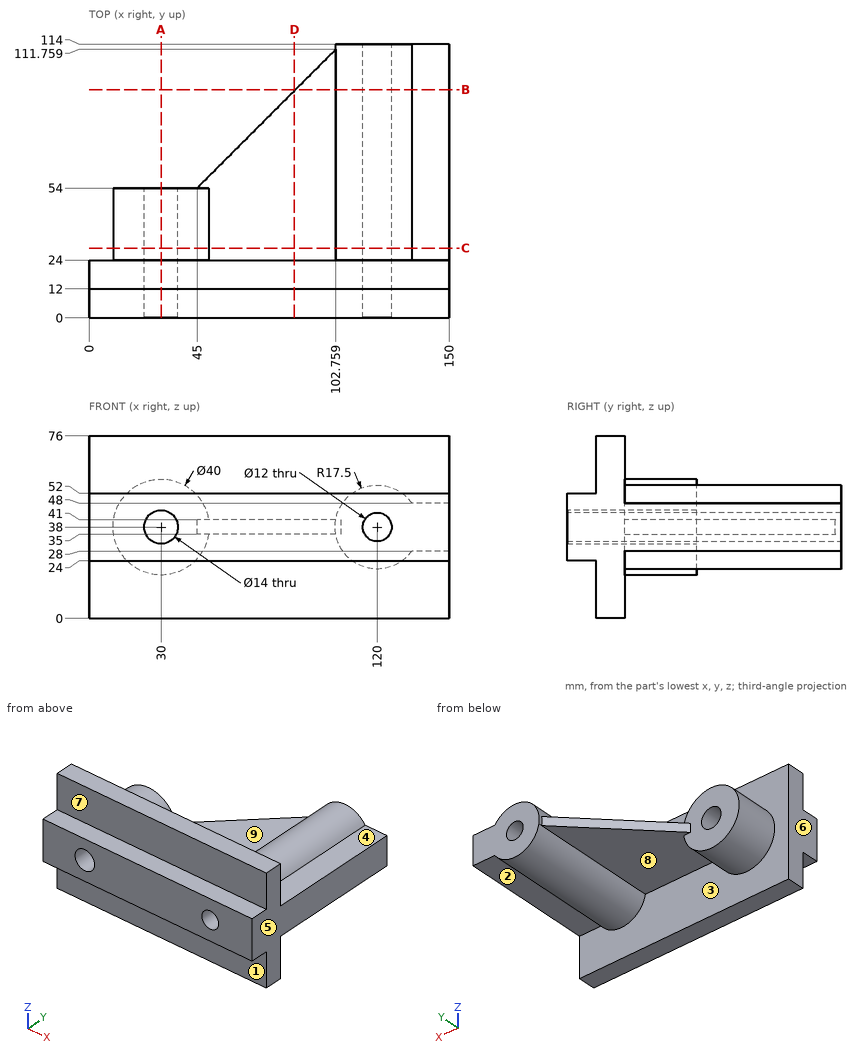
Could you check a few things on this drawing? It's one solid part, dimensions in mm from its lowest x, y, z. A direction names the side the tool comes from. Give positions to 0.01 mm unless a question says otherwise; leave off trailing zeros. Loops run counter-clockwise (first coordinate to the right, second up) from the corner with the lowest first, then second, coordinate; pieces in that order, holes last. Notation, with made-up numbers: M 3,56 L 42,56 A18 ccw 42,88 Z; hole C 2.5,-26 d6. An arc over 180 degrees is marked long. One line per question, with ' | ' between items. Start each with the question number.
Q1. If I drill on line 1 (X direction, y = 13, z = 38); line 2 (X direction, y = 30, z = 38); line 3 (X direction, y = 67, z = 38), over which ranges is the centre line in solid material (lowest first)? Write a range as from..to.
Q2. If we section it at C-C (y = 29): Please give me the cut outline in (x, z), plus the area to 3 significant figures.
Q3. For pin 1 Ø12 at (y, z) = (92.5, 20.5) entering from -X; pin 2 Ø17.5 at (x, y) = (73, 47.5) entering from +Z; pin 3 Ø19 at (x, z) = (93, 8.5) entering from -Y, each with a flat end and sliding along its axis, tell me the tip position at first contact or that it passes through.
Q4. If we section it at A-A (x = 30): Please give me the cut outline in (y, z), plus the area to 3 significant figures.
Q5. If we section it at D-D (x = 85.5): Please give me the cut outline in (y, z).
Q6. If we section it at B-B (y = 95): Please give me the cut outline in (x, z), plus the area to 3 significant figures.
Q7. If we mould it in two halves opening along X, with no side actions, what happens to the marked faces 6, 7, 8 and 9? For each: +X half, -X half, draft (parallel to the pull), parting line (faces both ways), or undercut.
Q8. For the marked faces 1, 2, 3, 4 and 5, which set-ups out of +Z, -Z, +X, -X, +Y, -Y let a thin tool reach every point of the face, with its end or its side?
Computed:
1) line 1: x = 0..23, 37..114, 126..150 | line 2: x = 10..23, 37..114, 126..150 | line 3: x = 58..114, 126..150
2) outline: M 49.77,35 L 102.76,35 A17.5 ccw 134.36,28 L 150,28 L 150,48 L 134.36,48 A17.5 ccw 102.76,41 L 49.77,41 A20 ccw long Z; hole C 30,38 d14; hole C 120,38 d12 | area: 2,540 mm²
3) pin 1: stops at x = 106.81 | pin 2: stops at z = 41 | pin 3: stops at y = 12
4) outline: M 0,24 L 12,24 L 12,0 L 24,0 L 24,18 L 54,18 L 54,31 L 0,31 Z; M 0,45 L 54,45 L 54,58 L 24,58 L 24,76 L 12,76 L 12,52 L 0,52 Z | area: 1,690 mm²
5) outline: M 0,24 L 12,24 L 12,0 L 24,0 L 24,35 L 94.5,35 L 94.5,41 L 24,41 L 24,76 L 12,76 L 12,52 L 0,52 Z
6) outline: M 86,35 L 102.76,35 A17.5 ccw 134.36,28 L 150,28 L 150,48 L 134.36,48 A17.5 ccw 102.76,41 L 86,41 Z; hole C 120,38 d12 | area: 1,220 mm²
7) face 6: -X half | face 7: draft | face 8: undercut | face 9: undercut
8) face 1: -Z, +X, -X, -Y | face 2: -Z, +X, +Y | face 3: +Y | face 4: +Z, +X, +Y | face 5: +Z, -Z, +X, +Y, -Y
